Could you check a few things on this model? Use its own coordinates, in mm. A direction names the side the tool comes from. Give positions to 0.01 mm unless a question says otherwise; leave off trailing zeros. Write each loop counter-clockwise with the first axis right and the second up, starting at its lowest first coordinate (ties: lowest second). Pieces come first, ordered by that corner, then holes. Notation, with made-up numbers: (-1, 61.25) - (38, 61.25) arc R16 cw to (38, 73.25) - close; hole circle Ø7 at (-26, 4.25). An arc over 180 degrees is marked (long way). Use one line per item in the form item = value.
```python
from build123d import *

# Parameters (mm, degrees)
EXTRUDE_1_DEPTH = 300
EXTRUDE_2_DEPTH = 10
EXTRUDE_3_DEPTH = 8
SKETCH_5_W      = 8
SKETCH_5_H      = 318
EXTRUDE_4_DEPTH = 8


with BuildPart() as part:
    # 草图1 → 凸台-拉伸1 (new body)
    with BuildSketch(Plane.XY):
        Polygon((0, 0), (0, 60), (-80, 60), (-80, 68), (8, 68), (8, 0), align=None)
    extrude(amount=EXTRUDE_1_DEPTH)

    # 草图2 → 凸台-拉伸2 (add)
    with BuildSketch(Plane.XY.offset(300)):
        Polygon((0, 0), (8, 0), (8, 68), (-80, 68), (-80, 60), (0, 60), align=None)
    extrude(amount=EXTRUDE_2_DEPTH)

    # 草图4 → 凸台-拉伸3 (add)
    with BuildSketch(Plane(origin=(0, 0, 0), x_dir=(-1, 0, 0), z_dir=(0, 0, -1))):
        Polygon((-8, 0), (0, 0), (0, 60), (80, 60), (80, 68), (-8, 68), align=None)
    extrude(amount=EXTRUDE_3_DEPTH)

    # 草图5 → 凸台-拉伸4 (add)
    with BuildSketch(Plane.XZ):
        with Locations((4, 151)):
            Rectangle(SKETCH_5_W, SKETCH_5_H)
    extrude(amount=EXTRUDE_4_DEPTH)


solid = part.part
```
1. Imagine slicing it at C-C, the plane y = 32.5. List the corners of the cut face in (x, z) for me, and give its area (3 significant figures).
Response values:
outline = (0, -8) - (8, -8) - (8, 310) - (0, 310) - close
area = 2,540 mm²
2. For pin 1 (3 mm diameter, centred on x = -30, z = 109.5, fed in from -Y); pin 2 (10 mm diameter, centred on x = -45, y = 57.5, fed in from -Z); pin 3 (3 mm diameter, centred on y = 39.5, z = 273.5, fed in from -X), each with a flat end and sliding along its axis, tell me the tip position at first contact or that it passes through.
Response values:
pin_1 = 60
pin_2 = -8
pin_3 = 0
3. Imagine slicing it at B-B, the plane x = -26. List the corners of the cut face in (y, z) for me.
Response values:
outline = (60, -8) - (68, -8) - (68, 310) - (60, 310) - close
4. If I drill on line 1 (Y direction, x = -37, z = 130.5); line 2 (X direction, y = 25, z = 15), over which ranges is the centre line in solid material (lowest first)? Write a range as from..to.
Response values:
line_1 = 60..68
line_2 = 0..8
5. Which directions (+Z, -Z, +X, -X, +Y, -Y) give clear straight access to the entire face, cutting with the end or side of a thin tool? Please do faces 1 (the face through (-20, 61, -8)), 2 (the face through (-39, 60, 153)).
Response values:
face_1 = -Z, +X, -X, +Y, -Y
face_2 = +Z, -Z, -X, -Y
6. Imagine slicing it at A-A, the plane z = 239. List the corners of the cut face in (x, y) for me.
Response values:
outline = (-80, 60) - (0, 60) - (0, -8) - (8, -8) - (8, 68) - (-80, 68) - close
